```python
from build123d import *

# Parameters (mm, degrees)
M3_TAPPED_HOLE1_D           = 2.5
M3_TAPPED_HOLE1_DEPTH       = 7
M3_TAPPED_HOLE1_CSINK_D     = 3.05
M3_TAPPED_HOLE1_CSINK_ANGLE = 90
M3_TAPPED_HOLE1_TIP         = 0.751075774


with BuildPart() as part:
    # Sketch1 → Revolve1 (revolve)
    with BuildSketch(Plane.XY, mode=Mode.PRIVATE) as revolve1_sk:
        Polygon((8.5, 0), (15.5, 0), (16, -0.5), (16, -8.5), (15.5, -9), (12, -9), (12, -9.2), (12.5, -9.7), (12.5, -15.7), (12.2, -16), (11, -16), (11, -17), (12, -17), (12, -22.5), (11.5, -23), (8.5, -23), (8, -22.5), (8, -0.5), align=None)
    revolve(revolve1_sk.sketch.rotate(Axis((0, 0, 0), (0, -1, 0)), 90), axis=Axis((0, 0, 0), (0, -1, 0)))

    # M3 Tapped Hole1
    with Locations(Plane(origin=(0, 0, 0), x_dir=(1, 0, 0), z_dir=(0, 1, 0))):
        with Locations((-12, 0), (0, 12), (12, 0), (0, -12)):
            CounterSinkHole(M3_TAPPED_HOLE1_D / 2, M3_TAPPED_HOLE1_CSINK_D / 2, depth=M3_TAPPED_HOLE1_DEPTH, counter_sink_angle=M3_TAPPED_HOLE1_CSINK_ANGLE)
            with Locations((0, 0, -(M3_TAPPED_HOLE1_DEPTH + M3_TAPPED_HOLE1_TIP / 2))):  # 118° drill point
                Cone(0, M3_TAPPED_HOLE1_D / 2, M3_TAPPED_HOLE1_TIP, mode=Mode.SUBTRACT)


solid = part.part
```
Verification items for the finished model (mm, model axes). A direction names the side the tool comes from. Coordinates: 2 decimals unless noted, no trailing zeros. Order: outer loops, then holes, each group sorted by start corner. A loop starts at its lowest first (then second) coordinate and runs counter-clockwise, first axis right, second up. Notation, with made-up numbers: (6.5, -25) - (60.5, -25) arc R29 ccw to (60.5, -2) - close; hole circle Ø11 at (-26, 87.25). An arc over 180 degrees is marked (long way). Return JSON: item names as keys, results as strings.
(1) Thickness scan on line 1 along Y through (x, z) = (-11, 3); line 2 along Y through (x, z) = (-11.5, 9.5); line 3 along X through (y, z) = (-11, -3.5). Record the ranges inside material, lowest first.
Filled sheet:
{"line 1": "y = -23 to -17, -16 to 0", "line 2": "y = -9 to 0", "line 3": "x = -12 to -7.19, 7.19 to 12"}
(2) Section check A-A, the plane y = -19.75. Record the cut outline in (x, z).
Filled sheet:
{"outline": "circle Ø24 at (0, 0); hole circle Ø16 at (0, 0)"}
(3) Go/stop test with flat-tipped pins: pin 1 (7.5 mm diameter, centred on x = 1.5, z = -3.5, fed in from -Y); pin 2 (1.5 mm diameter, centred on y = -6, z = -3.5, fed in from -X); pin 3 (5 mm diameter, centred on x = 1.5, z = 5.5, fed in from +Y); pin 4 (1.5 mm diameter, centred on y = -9.5, z = -10, fed in from +X). Record where each tip stops, or that it passes through.
Filled sheet:
{"pin 1": "passes through", "pin 2": "stops at x = -15.76", "pin 3": "stops at y = -0.3", "pin 4": "stops at x = 12.34"}
(4) Mould release check, pull along Z, two halves, no side actions. Record for faces 5 (the cylindrical face through (0.16, -3.68, 10.76)), 6 (the flat face through (11.4, -9, 4.5)), 7 (the cylindrical face through (-3.755, -12.742, 11.923)): pulls with the +Z half, pulls with the -Z half, needs draft (parallel to the pull), parting line crosses it, or undercut.
Filled sheet:
{"face 5": "undercut", "face 6": "needs draft", "face 7": "parting line crosses it"}
(5) Access from +Z, -Z, +X, -X, +Y, -Y to the whole of each face (thin tool, end or side, straight path). Record for faces 1 (the cylindrical face through (-3.604, -19.788, 11.446)), 2 (the cylindrical face through (-10.75, -3.68, -0.05)), 3 (the cylindrical face through (15.62, -4.56, -3.47)), 4 (the flat face through (10, -17, -5)).
Filled sheet:
{"face 1": "-Y", "face 2": "+Y", "face 3": "+Y, -Y", "face 4": "none"}
